Could you check a few things on this drawing? It's one solid part, dimensions in mm from its lowest x, y, z. Give positions to 0.01 mm unless a question says otherwise; leave off trailing zeros. Loops run counter-clockwise (first coordinate to the right, second up) from the corner with the lowest first, then second, coordinate; pieces in that order, holes last. Notation, with made-up numbers: (26, -19.5) - (32, -19.5) arc R30 ccw to (32, 8.5) - close; hole circle Ø9 at (1, 79). An arc over 180 degrees is marked (long way). Return JSON: item names as keys, results as strings. Group by question number.
(1) If we section it at A-A (z = 1.5): Please give me the cut outline in (x, y).
(2) I need wall thicknesses on probe 1 along X at (y, z) = (72.5, 5); probe 2 along Y at (x, z) = (35, 4); probe 3 along X at (y, z) = (67.5, 0.5). Which ranges of each line are inside material? Lowest first, please. Write a range as [from, to].
(3) For P1, Ø4, axis at x = 364, z = 6, coming from the -Y side, with a flat end and sliding along its axis, tell me the tip position at first contact or that it passes through.
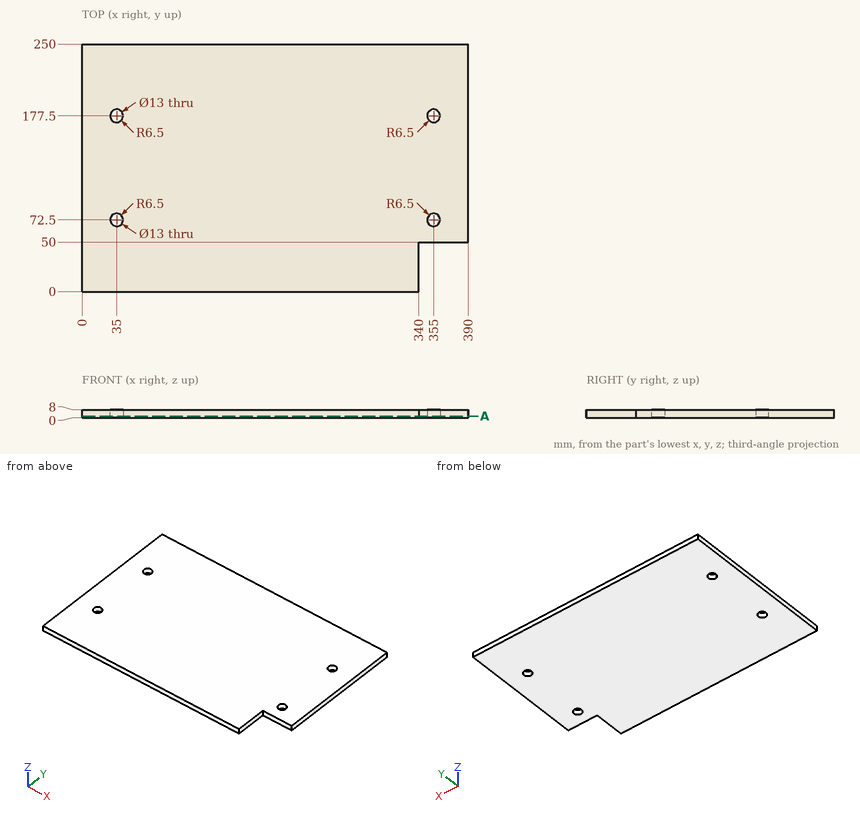
Values:
{
 "1": {"outline": "(0, 0) - (340, 0) - (340, 50) - (390, 50) - (390, 250) - (0, 250) - close; hole circle Ø13 at (35, 72.5); hole circle Ø13 at (35, 177.5); hole circle Ø13 at (355, 72.5); hole circle Ø13 at (355, 177.5)"},
 "2": {"probe 1": "[0, 28.5], [41.5, 348.5], [361.5, 390]", "probe 2": "[0, 66], [79, 171], [184, 250]", "probe 3": "[0, 30.85], [39.15, 350.85], [359.15, 390]"},
 "3": {"P1": "y = 50"}
}
